The listing builds one solid part. Answer for the finished solid, in the listing's coordinates (mm). Face numbers are marked on the shaded views. A direction names the side the tool comes from. Give positions to 0.01 mm unless a question says otherwise; leave off trailing zeros. Order: outer loops, then holes, each group sorted by start corner. A loop starts at its lowest first (then second) coordinate and runs counter-clockwise, first axis right, second up. Notation, with made-up numbers: (11, 60) - (70, 60) arc R9 ccw to (70, 68) - close; hole circle Ø11 at (82.5, 89). An arc over 180 degrees is marked (long way). Answer in a Markdown table with one row per item.
from build123d import *

# Parameters (mm, degrees)
ROD_PROFILE_SKETCH_R         = 5
ROD_PROFILE_SKETCH_R_2       = 3
ROD_BODY_EXTRUDE_8MM_DEPTH   = 4
ROD_PROFILE_SKETCH_R_3       = 7.5
ROD_BODY_EXTRUDE_8MM_2_DEPTH = 4
SHANK_BOSS_4MM_DEPTH         = 2
SHANK_FILLET_R2_R            = 2


with BuildPart() as part:
    # Rod Profile Sketch → Rod Body Extrude 8mm (new, symmetric)
    with BuildSketch(Plane.XY):
        with Locations((-29.25, 0)):
            Circle(ROD_PROFILE_SKETCH_R)
        with Locations((-29.25, 0)):
            Circle(ROD_PROFILE_SKETCH_R_2, mode=Mode.SUBTRACT)
    extrude(amount=ROD_BODY_EXTRUDE_8MM_DEPTH, both=True)



with BuildPart() as body_2:
    # Rod Profile Sketch → Rod Body Extrude 8mm 2 (new, symmetric)
    with BuildSketch(Plane.XY):
        with Locations((26.75, 0)):
            Circle(ROD_PROFILE_SKETCH_R_3)
        with Locations((26.75, 0)):
            Circle(ROD_PROFILE_SKETCH_R, mode=Mode.SUBTRACT)
    extrude(amount=ROD_BODY_EXTRUDE_8MM_2_DEPTH, both=True)


with BuildPart() as part_1:
    add(part.part)

    add(body_2.part)  # Shank Boss 4mm merges body 2
    # Shank Boss Sketch → Shank Boss 4mm (add, symmetric)
    with BuildSketch(Plane.XY):
        with BuildLine():
            Line((-24.667424305, 2), (19.521583853, 2))
            ThreePointArc((19.521583853, 2), (19.25, 0), (19.521583853, -2))
            Line((19.521583853, -2), (-24.667424305, -2))
            ThreePointArc((-24.667424305, -2), (-24.25, 0), (-24.667424305, 2))
        make_face()
    extrude(amount=SHANK_BOSS_4MM_DEPTH, both=True)

    # Shank Fillet R2
    shank_fillet_r2_edges = [part_1.edges().sort_by_distance(p)[0] for p in [
        (19.521583853, -2, 0),
        (19.521583853, 2, 0),
        (-24.667424305, 2, 0),
        (-24.667424305, -2, 0),
    ]]
    fillet(shank_fillet_r2_edges, radius=SHANK_FILLET_R2_R)


solid = part_1.part
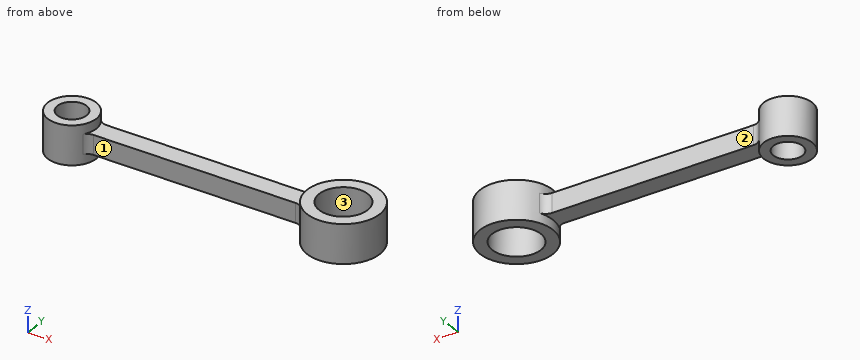
Item 1: Which of the six approach directions +Z, -Z, +X, -X, +Y, -Y give full straight-line access (tool end or side, diameter ignored) to the marked faces 1, 2 and 3?
Answer block:
| item | result |
|---|---|
| face 1 | +Z, -Z, -Y |
| face 2 | +Z, -Z, +Y |
| face 3 | +Z, -Z |
Item 2: Find section C-C on z = -3. Write down the section's boundary in (x, y), then the cut area to 3 significant figures.
Answer block:
| item | result |
|---|---|
| outline | circle Ø10 at (-29.25, 0); circle Ø15 at (26.75, 0); hole circle Ø6 at (-29.25, 0); hole circle Ø10 at (26.75, 0) |
| area | 148 mm² |
Item 3: Consider line 1 (Y direction, x = 26.75, z = 2.5); line 2 (X direction, y = -2.5, z = 1); line 3 (Y direction, x = -29.25, z = 1.5). Determine where each line is inside the solid, lowest interval first.
Answer block:
| item | result |
|---|---|
| line 1 | -7.5 to -5, 5 to 7.5 |
| line 2 | -33.58 to -30.91, -27.59 to -24.83, 19.46 to 22.42, 31.08 to 33.82 |
| line 3 | -5 to -3, 3 to 5 |
Item 4: Find section A-A on x = 26.75. Write down the section's boundary in (y, z).
Answer block:
| item | result |
|---|---|
| outline | (-7.5, -4) - (-5, -4) - (-5, 4) - (-7.5, 4) - close; (5, -4) - (7.5, -4) - (7.5, 4) - (5, 4) - close |
Item 5: Find section D-D on z = -0.5. Write down the section's boundary in (x, y), then the cut area to 3 significant figures.
Answer block:
| item | result |
|---|---|
| outline | (-25.15, -2.86) arc R2 cw to (-23.51, -2) - (18.13, -2) arc R2 cw to (19.95, -3.16) arc R7.5 ccw (long way) to (19.95, 3.16) arc R2 cw to (18.13, 2) - (-23.51, 2) arc R2 cw to (-25.15, 2.86) arc R5 ccw (long way) to start; hole circle Ø6 at (-29.25, 0); hole circle Ø10 at (26.75, 0) |
| area | 324 mm² |
Item 6: Each of these flat-tipped pins is pushed along its axis until it touches: P1, Ø6, axis at x = -7.5, y = -3.5, coming from the +Z side; P2, Ø1.5, axis at x = -2, y = -2, coming from the -Z side; P3, Ø7, axis at x = -29.25, y = 0, coming from the +Z side; P4, Ø1.5, axis at x = -9.5, z = -3, coming from the +Y side. Where does it stop, or does it pass through?
Answer block:
| item | result |
|---|---|
| P1 | z = 2 |
| P2 | z = -2 |
| P3 | z = 4 |
| P4 | through |
Item 7: Find section B-B on y = 0. Write down the section's boundary in (x, z), then the cut area to 3 significant figures.
Answer block:
| item | result |
|---|---|
| outline | (-34.25, -4) - (-32.25, -4) - (-32.25, 4) - (-34.25, 4) - close; (-26.25, -4) - (-24.25, -4) - (-24.25, -2) - (19.25, -2) - (19.25, -4) - (21.75, -4) - (21.75, 4) - (19.25, 4) - (19.25, 2) - (-24.25, 2) - (-24.25, 4) - (-26.25, 4) - close; (31.75, -4) - (34.25, -4) - (34.25, 4) - (31.75, 4) - close |
| area | 246 mm² |
